The model under review builds one solid part; all positions refer to its coordinate system, in mm. Face numbers are marked on the shaded views. A direction names the side the tool comes from. Coordinates: 2 decimals unless noted, no trailing zeros. Order: outer loops, then holes, each group sorted by start corner. A loop starts at its lowest first (then second) coordinate and runs counter-clockwise, first axis right, second up. Notation, with made-up numbers: M 67.5,0 L 82.5,0 A27 ccw 82.5,24 Z; hole C -30.75,-3 d2. An arc over 180 degrees is marked long. One line per item, written item: value.
```python
from build123d import *

# Parameters (mm, degrees)
DISC_PROFILE_R        = 47.5
DISC_95X5_DEPTH       = 5
DRIVE_PIN_PROFILE_R   = 5.3
DRIVE_PIN_10_6_DEPTH  = 10
HUB_PROFILE_R         = 27
HUB_54X10_DEPTH       = 10
HUB_START             = -10
HUB_FLAT_CUT_DEPTH    = 10
CENTRE_BORE_PROFILE_R = 5
CENTRE_BORE_10_DEPTH  = 30


with BuildPart() as part:
    # Disc Profile → Disc Ø95x5 (new body)
    with BuildSketch(Plane.XY):
        Circle(DISC_PROFILE_R)
    extrude(amount=DISC_95X5_DEPTH)

    # Drive Pin Profile → Drive Pin Ø10.6 (add)
    with BuildSketch(Plane.XY.offset(5)):
        with Locations((-39, 0)):
            Circle(DRIVE_PIN_PROFILE_R)
    extrude(amount=DRIVE_PIN_10_6_DEPTH)

    # Hub Profile → Hub Ø54x10 (add)
    with BuildSketch(Plane.XY.offset(5)):
        Circle(HUB_PROFILE_R)
    extrude(amount=HUB_54X10_DEPTH)

    # Hub Flat Profile → Hub Flat Cut (cut)
    with BuildSketch(Plane.XY.offset(15).offset(HUB_START)):
        with BuildLine():
            ThreePointArc((-22.179240987, 15.397443595), (-27, 0), (-22.179240987, -15.397443595))
            ThreePointArc((-22.179240987, -15.397443595), (-17.358481974, 0), (-22.179240987, 15.397443595))
        make_face()
    extrude(amount=HUB_FLAT_CUT_DEPTH, mode=Mode.SUBTRACT)

    # Centre Bore Profile → Centre Bore Ø10 (cut)
    with BuildSketch(Plane.XY.offset(15)):
        Circle(CENTRE_BORE_PROFILE_R)
    extrude(amount=-CENTRE_BORE_10_DEPTH, mode=Mode.SUBTRACT)


solid = part.part
```
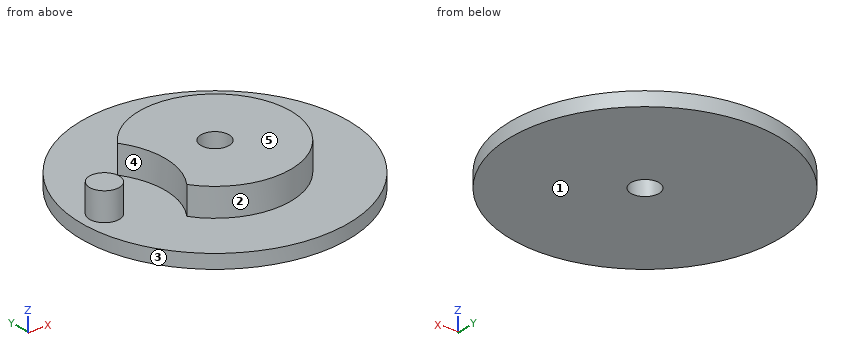
(1) For L1, parallel to Y at x = 0, z = 10; L2, parallel to Y at x = 0, z = 4.5; L3, parallel to Z at x = -14, y = -34.5, list the stretches that pass through material, from the lowest coordinate up.
Geometry results:
L1: y = -27 to -5, 5 to 27
L2: y = -47.5 to -5, 5 to 47.5
L3: z = 0 to 5
(2) We need section A-A, the plane y = 0. State the section outline as (x, z) points.
Geometry results:
outline: M -47.5,0 L -5,0 L -5,15 L -17.36,15 L -17.36,5 L -33.7,5 L -33.7,15 L -44.3,15 L -44.3,5 L -47.5,5 Z; M 5,0 L 47.5,0 L 47.5,5 L 27,5 L 27,15 L 5,15 Z
(3) We need section C-C, the plane z = 12. State the section outline as (x, y) points.
Geometry results:
outline: C -39,0 d10.6; M -22.18,-15.4 A27 ccw long -22.18,15.4 A27 cw Z; hole C 0,0 d10
(4) Mouldability with a two-part tool opening along X and no side actions: class the marked faces 3, 4 and 5 as +X half, -X half, draft (parallel to the pull), parting line (faces both ways), or undercut.
Geometry results:
face 3: parting line
face 4: undercut
face 5: draft
(5) We need section B-B, the plane x = -1. State the section outline as (y, z) points.
Geometry results:
outline: M -47.49,0 L -4.9,0 L -4.9,15 L -26.98,15 L -26.98,5 L -47.49,5 Z; M 4.9,0 L 47.49,0 L 47.49,5 L 26.98,5 L 26.98,15 L 4.9,15 Z
(6) Tool access review of the marked faces 1 and 2: name each direction out of +Z, -Z, +X, -X, +Y, -Y from which nothing blocks a thin tool from reaching the whole face with its end or side.
Geometry results:
face 1: -Z, +X, -X, +Y, -Y
face 2: +Z
(7) We need section D-D, the plane x = -39. State the section outline as (y, z) points.
Geometry results:
outline: M -27.12,0 L 27.12,0 L 27.12,5 L 5.3,5 L 5.3,15 L -5.3,15 L -5.3,5 L -27.12,5 Z
(8) Insertion check: pin 1 Ø5 at (x, z) = (9.5, 11.5) entering from +Y; pin 2 Ø8 at (y, z) = (31, 7.5) entering from +X; pin 3 Ø2 at (y, z) = (14, 13) entering from +X; pin 4 Ø1 at (x, z) = (-26, 7) entering from -Y. Each pin has a flat end and moves straight along its axis. Give the tip position at first contact, or say it passes through.
Geometry results:
pin 1: stops at y = 26.08
pin 2: stops at x = 38.46
pin 3: stops at x = 23.66
pin 4: passes through
